The model under review builds one solid part; all positions refer to its coordinate system, in mm. Face numbers are marked on the shaded views. A direction names the side the tool comes from. Give positions to 0.01 mm unless a question says otherwise; leave off trailing zeros. Write each loop counter-clockwise with the first axis right and the second up, starting at its lowest first coordinate (ties: lowest second). Pieces come first, ordered by that corner, then holes.
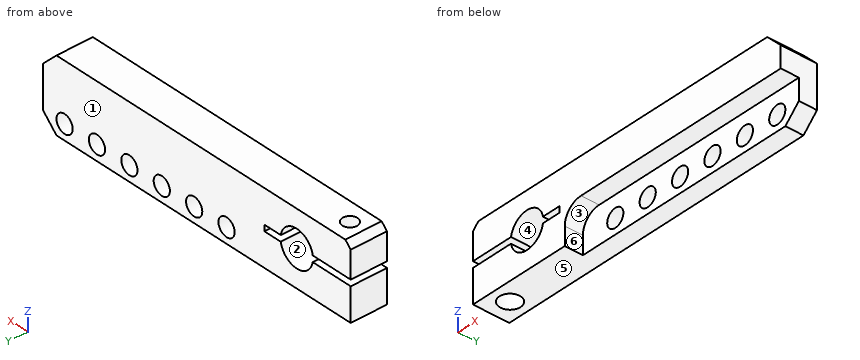
from build123d import *

# Parameters (mm, degrees)
SKETCH1_W                = 65
SKETCH1_H                = 12
SKETCH1_R                = 3
BOSS_EXTRUDE1_DEPTH      = 6
SKETCH2_W                = 32
SKETCH2_H                = 1
CUT_EXTRUDE1_DEPTH       = 34.589432862
SKETCH4_R                = 1.75
CUT_EXTRUDE3_DEPTH       = 6
M3_TAPPED_HOLE1_D        = 2.5
SKETCH10_W               = 48
SKETCH10_H               = 6
CUT_EXTRUDE4_DEPTH       = 3
F_3_0_3_DIAMETER_HOLE1_D = 3
LPATTERN1_COUNT          = 6
LPATTERN1_PITCH          = 6
FILLET1_R                = 3
SKETCH11_W               = 8
SKETCH11_H               = 12
CUT_EXTRUDE5_DEPTH       = 10
CHAMFER1_SIZE            = 1
CHAMFER2_SIZE            = 2.5


with BuildPart() as part:
    # Sketch1 → Boss-Extrude1 (new body)
    with BuildSketch(Plane(origin=(0, 0, 0), x_dir=(1, 0, 0), z_dir=(0, 1, 0))):
        Rectangle(SKETCH1_W, SKETCH1_H)
        with Locations(Location((-22.5, 0, 0), (0, 0, 270))):
            Circle(SKETCH1_R, mode=Mode.SUBTRACT)
    extrude(amount=BOSS_EXTRUDE1_DEPTH)

    # Sketch2 → Cut-Extrude1 (cut, through all)
    with BuildSketch(Plane.XZ):
        with Locations((-32.5, 0)):
            Rectangle(SKETCH2_W, SKETCH2_H)
    extrude(amount=-CUT_EXTRUDE1_DEPTH, mode=Mode.SUBTRACT)

    # Sketch4 → Cut-Extrude3 (cut)
    with BuildSketch(Plane(origin=(0, 0, -6), x_dir=(-1, 0, 0), z_dir=(0, 0, -1))):
        with Locations((29, 3)):
            Circle(SKETCH4_R)
    extrude(amount=-CUT_EXTRUDE3_DEPTH, mode=Mode.SUBTRACT)

    # M3 Tapped Hole1 (through all)
    with Locations(Plane(origin=(-29, 3, 0.5), x_dir=(-1, 0, 0), z_dir=(0, 0, -1))):
        with Locations((0, 0)):
            Hole(M3_TAPPED_HOLE1_D / 2)

    # Sketch10 → Cut-Extrude4 (cut)
    with BuildSketch(Plane.XZ):
        with Locations((8.5, -3)):
            Rectangle(SKETCH10_W, SKETCH10_H)
    extrude(amount=-CUT_EXTRUDE4_DEPTH, mode=Mode.SUBTRACT)

    # Ø3.0 (3) Diameter Hole1 (through all)
    with Locations(Plane(origin=(20.5, 0, -3.5), x_dir=(0, 0, -1), z_dir=(0, -1, 0))):
        with Locations((0, 0)):
            f_3_0_3_diameter_hole1 = Hole(F_3_0_3_DIAMETER_HOLE1_D / 2)

    # LPattern1: Ø3.0 (3) Diameter Hole1 ×6
    with Locations(*[(-i * LPATTERN1_PITCH, 0, 0) for i in range(1, LPATTERN1_COUNT)]):
        add(f_3_0_3_diameter_hole1, mode=Mode.SUBTRACT)

    # Fillet1
    fillet1_edges = [part.edges().sort_by_distance(p)[0] for p in [
        (-15.5, 1.5, 0),
    ]]
    fillet(fillet1_edges, radius=FILLET1_R)

    # Sketch11 → Cut-Extrude5 (cut)
    with BuildSketch(Plane.XZ):
        with Locations((28.5, 0)):
            Rectangle(SKETCH11_W, SKETCH11_H)
    extrude(amount=-CUT_EXTRUDE5_DEPTH, mode=Mode.SUBTRACT)

    # Chamfer1
    chamfer1_edges = [part.edges().sort_by_distance(p)[0] for p in [
        (-32.5, 3, 6),
    ]]
    chamfer(chamfer1_edges, length=CHAMFER1_SIZE)

    # Chamfer2
    chamfer2_edges = [part.edges().sort_by_distance(p)[0] for p in [
        (24.5, 4.5, -6),
        (24.5, 3, 6),
    ]]
    chamfer(chamfer2_edges, length=CHAMFER2_SIZE)


solid = part.part
1) Tool access review of the marked faces 5 and 6: name each direction out of +Z, -Z, +X, -X, +Y, -Y from which nothing blocks a thin tool from reaching the whole face with its end or side.
2) Insertion check: pin 1 (3 mm diameter, centred on x = -12, z = -4.5, fed in from -Y); pin 2 (1.5 mm diameter, centred on y = 1, z = -4.5, fed in from +X). Each pin has a flat end and moves straight along its axis. Give the tip position at first contact, or say it passes through.
3) Consider section A-A, the plane x = 20.5. Give the boundary of the cut face in (y, z), then the cut area to 3 significant figures.
4) To check wall thickness, follow probe 1 along X at (y, z) = (2.9, 1.25); probe 2 along Z at (x, y) = (-18, 5); probe 3 along Y at (x, z) = (17.5, -2.25). State the ranges of each line that lie inside material, in increasing order.
5) Consider section B-B, the plane x = -29. Give the boundary of the cut face in (y, z).
6) Consider section D-D, the plane y = 2.25. Give the boundary of the cut face in (x, z), then the cut area to 3 significant figures.
7) The part is to be moulded in two halves that separate along Z. For the marked faces 1, 2, 3 and 4, say which applies: +Z half, -Z half, draft (parallel to the pull), parting line (faces both ways), or undercut.
8) Consider section C-C, the plane z = -1. Give the boundary of the cut face in (x, y), then the cut area to 3 significant figures.
Answer block:
1. face 5: -Z, +X, -X, +Y, -Y
1. face 6: -Z, +X, -Y
2. pin 1: stops at y = 3
2. pin 2: stops at x = -15.5
3. outline: (0, 0) - (3, 0) - (3, -2) - (6, -2) - (6, 6) - (0, 6) - close; (3, -6) - (6, -6) - (6, -5) - (3, -5) - close
3. area: 45.0 mm2
4. probe 1: x = -32.5 to -30.25, -27.75 to -25.23, -19.77 to 24.5
4. probe 2: z = -6 to -0.5, 0.5 to 6
4. probe 3: y = 3 to 6
5. outline: (0, -6) - (1.25, -6) - (1.25, -0.5) - (0, -0.5) - close; (0, 0.5) - (1.75, 0.5) - (1.75, 6) - (0, 6) - close; (4.25, 0.5) - (6, 0.5) - (6, 6) - (4.25, 6) - close; (4.75, -6) - (6, -6) - (6, -0.5) - (4.75, -0.5) - close
6. outline: (-32.5, -6) - (-30.58, -6) - (-30.58, -0.5) - (-32.5, -0.5) - close; (-32.5, 0.5) - (-30, 0.5) - (-30, 6) - (-31.5, 6) - (-32.5, 5) - close; (-28, 0.5) - (-25.46, 0.5) arc R3 cw to (-19.54, 0.5) - (-16.5, 0.5) - (-16.5, -0.5) - (-19.54, -0.5) arc R3 cw to (-25.46, -0.5) - (-27.42, -0.5) - (-27.42, -6) - (-15.5, -6) - (-15.5, -3) arc R3 cw to (-12.5, 0) - (24.5, 0) - (24.5, 3.5) - (22, 6) - (-28, 6) - close
6. area: 376 mm2
7. face 1: draft
7. face 2: undercut
7. face 3: -Z half
7. face 4: undercut
8. outline: (-32.5, 0) - (-25.33, 0) - (-25.33, 6) - (-32.5, 6) - close; (-19.67, 0) - (-14.74, 0) - (-14.74, 3) - (24.5, 3) - (24.5, 6) - (-19.67, 6) - close; hole circle Ø3.5 at (-29, 3)
8. area: 181 mm2
